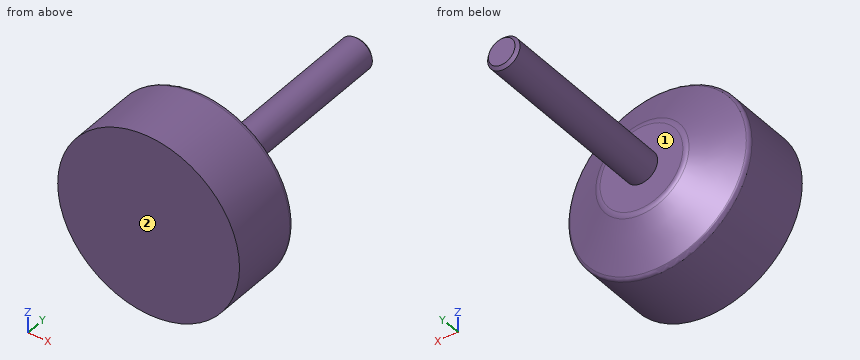
```python
from build123d import *


with BuildPart() as part:
    # 草图1 → 旋转1 (revolve)
    with BuildSketch(Plane(origin=(0, 0, 0), x_dir=(-1, 0, 0), z_dir=(0, 0, -1)), mode=Mode.PRIVATE) as revolve_1_sk:
        with BuildLine():
            Line((-20, -25), (-0.54, -25))
            Line((-0.54, -25), (-0.54, 35))
            Line((-0.54, 35), (-3.3865, 35))
            Line((-3.3865, 35), (-4, 34.3865))
            Line((-4, 34.3865), (-4, -5))
            Line((-4, -5), (-9.409830056, -5))
            ThreePointArc((-9.409830056, -5), (-9.984212358, -5.066877526), (-10.527864045, -5.263932023))
            Line((-10.527864045, -5.263932023), (-19.447213595, -9.723606798))
            ThreePointArc((-19.447213595, -9.723606798), (-19.850650808, -10.092302877), (-20, -10.618033989))
            Line((-20, -10.618033989), (-20, -25))
        make_face()
    revolve(revolve_1_sk.sketch.rotate(Axis((0.54, -25, 0), (0, 1, 0)), 180), axis=Axis((0.54, -25, 0), (0, 1, 0)))


solid = part.part
```
Could you check a few things on this model? Use its own coordinates, in mm. Face numbers are marked on the shaded views. A direction names the side the tool comes from. Round coordinates to 2 decimals unless told otherwise and drop trailing zeros. Write each loop counter-clockwise with the first axis right and the second up, starting at its lowest first coordinate (ties: lowest second). Pieces come first, ordered by that corner, then holes. Notation, with made-up numbers: M 80,63.5 L 131,63.5 A31 cw 131,96.5 Z; hole C -5.75,-16 d8. An arc over 180 degrees is marked long. Write each question's results on one line, items separated by ' | '. Start each with the question number.
1. Imagine slicing it at A-A on x = 0.54. List the corners of the cut face in (y, z) for me.
2. On a 3-axis mill with a long thin cutter (end or side, diameter ignored), from which of +Z, -Z, +X, -X, +Y, -Y can I reach the whole of each face in a straight line? I mean the marked faces 1 and 2. Say none if no direction works.
3. I'm going to push flat-ended pins straight in: pin 1 Ø12 at (y, z) = (6.5, 6.5) entering from +X; pin 2 Ø5 at (y, z) = (18.5, -7.5) entering from -X; pin 3 Ø3 at (x, y) = (-4, 16.5) entering from -Z; pin 4 Ø5 at (y, z) = (-11.5, -5) entering from +X. Where does each tip first touch, or does it pass through?
4. Imagine slicing it at B-B on z = 0. List the corners of the cut face in (x, y) for me.
5. I need wall thicknesses on L1, parallel to Y at x = 8.5, z = 17; L2, parallel to X at y = -11, z = 8; L3, parallel to Y at x = 11.5, z = 11. Which ranges of each line are inside material? Lowest first, please. Write a range as from..to.
6. Imagine slicing it at C-C on y = 9. List the corners of the cut face in (x, z) for me.
Result sheet:
1) outline: M -25,-19.46 L -10.62,-19.46 A1 ccw -9.72,-18.91 L -5.26,-9.99 A2.5 ccw -5,-8.87 L -5,-3.46 L 34.39,-3.46 L 35,-2.85 L 35,2.85 L 34.39,3.46 L -5,3.46 L -5,8.87 A2.5 ccw -5.26,9.99 L -9.72,18.91 A1 ccw -10.62,19.46 L -25,19.46 Z
2) face 1: +Y | face 2: +Z, -Z, +X, -X, -Y
3) pin 1: stops at x = 3.96 | pin 2: passes through | pin 3: stops at z = -1.65 | pin 4: stops at x = 19.84
4) outline: M -18.92,-25 L 20,-25 L 20,-10.62 A1 ccw 19.45,-9.72 L 10.53,-5.26 A2.5 ccw 9.41,-5 L 4,-5 L 4,34.39 L 3.39,35 L -2.31,35 L -2.92,34.39 L -2.92,-5 L -8.33,-5 A2.5 ccw -9.45,-5.26 L -18.37,-9.72 A1 ccw -18.92,-10.62 Z
5) L1: y = -25..-9.66 | L2: x = -17.2..18.28 | L3: y = -25..-8.03
6) outline: C 0.54,0 d6.92
